Geometry: see drawing. Coordinates: mm, zero at the bounding-box minimum. Coordinates: 2 decimals unless noted, no trailing zeros. Order: outer loops, then holes, each group sorted by start corner. A loop starts at its lowest first (then second) coordinate and runs counter-clockwise, first axis right, second up. Notation, with made-up numbers: (-14, -13) - (-9, -13) arc R24 ccw to (-9, 0) - close; hole circle Ø3 at (85.25, -6). An arc over 180 degrees is marked (long way). Use a Markdown table: item, result. Add a question column.
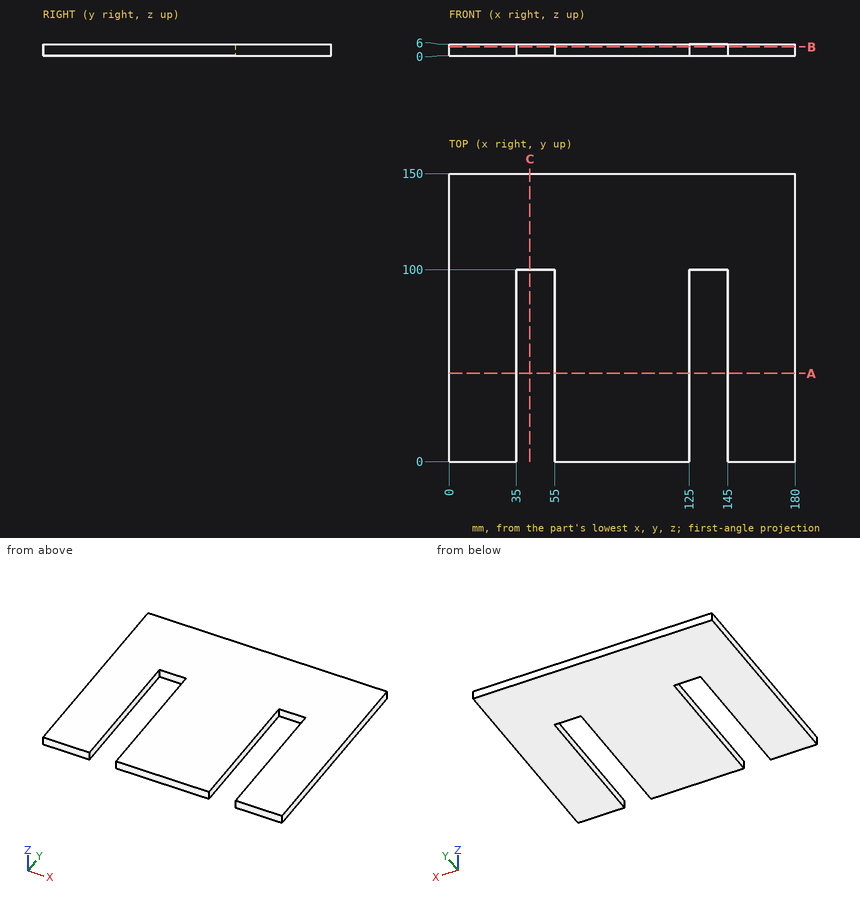
1) First-contact query: pin 1 (1 mm diameter, centred on y = 36.5, z = 4.5, fed in from -X); pin 2 (3 mm diameter, centred on x = 40.5, z = 2.5, fed in from -Y). Flat tips, straight axial feed; report the tip coordinate or a pass-through.
2) Section query B-B (z = 4.55). Return the cut outline in (x, y), and give its area (3 significant figures).
3) Section query C-C (x = 42). Return the cut outline in (y, z), and give its area (3 significant figures).
4) Section query A-A (y = 46). Return the cut outline in (x, z), and give its area (3 significant figures).
5) Line query: line 1 (X direction, y = 89, z = 3.2); line 2 (Y direction, x = 141, z = 2.4). Output: solid intervals per line, ascending. Write a range as from..to.
From the geometry:
| question | item | result |
|---|---|---|
| 1 | pin 1 | stops at x = 0 |
| 1 | pin 2 | stops at y = 100 |
| 2 | outline | (0, 0) - (35, 0) - (35, 100) - (55, 100) - (55, 0) - (125, 0) - (125, 100) - (145, 100) - (145, 0) - (180, 0) - (180, 150) - (0, 150) - close |
| 2 | area | 23,000 mm^2 |
| 3 | outline | (100, 0) - (150, 0) - (150, 6) - (100, 6) - close |
| 3 | area | 300 mm^2 |
| 4 | outline | (0, 0) - (35, 0) - (35, 6) - (0, 6) - close; (55, 0) - (125, 0) - (125, 6) - (55, 6) - close; (145, 0) - (180, 0) - (180, 6) - (145, 6) - close |
| 4 | area | 840 mm^2 |
| 5 | line 1 | x = 0..35, 55..125, 145..180 |
| 5 | line 2 | y = 100..150 |
